Design review of the part built by this model. Coordinates are the model's own, in mm. Coordinates: 2 decimals unless noted, no trailing zeros.
Q1. Take a section at A-A, the plane z = 4. State how many separate pieces and enclosed holes the cut face has, plus the area to 3 significant figures.
Q2. For pin 1 Ø5 at (x, y) = (0, 70.5) entering from -Z, flat-tipped, find the tip position at first contact; note if it passes through.
Q3. For L1, parallel to Y at x = 98, z = 0.9, list the stretches that pass through material, from the lowest coordinate up.
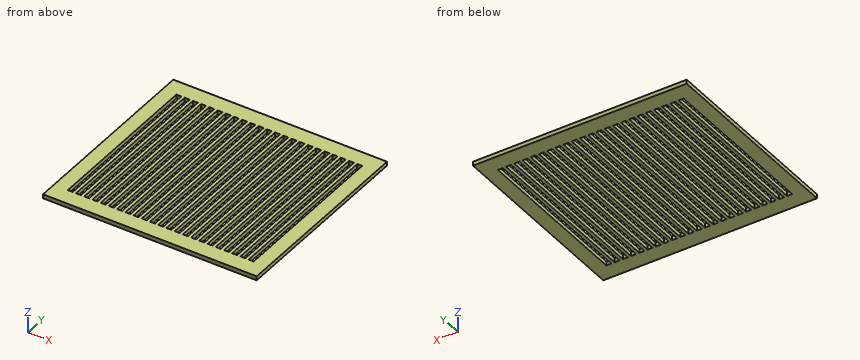
from build123d import *

# Parameters (mm, degrees)
SKETCH_1_W                 = 260
SKETCH_1_H                 = 240
EXTRUDE_1_DEPTH            = 5
SKETCH_2_W                 = 6
SKETCH_2_H                 = 200
CUT_EXTRUDE_1_DEPTH        = 177.988700204
PATTERN_LINEAR_1_COUNT     = 12
PATTERN_LINEAR_1_PITCH     = 10
PATTERN_LINEAR_1_COL_COUNT = 12
PATTERN_LINEAR_1_COL_PITCH = 10


with BuildPart() as part:
    # 草图1 → 凸台-拉伸1 (new body)
    with BuildSketch(Plane.XY):
        Rectangle(SKETCH_1_W, SKETCH_1_H)
    extrude(amount=EXTRUDE_1_DEPTH)

    # 草图2 → 切除-拉伸1 (cut, through all)
    with BuildSketch(Plane.XY.offset(5)):
        Rectangle(SKETCH_2_W, SKETCH_2_H)
    cut_extrude_1 = extrude(amount=-CUT_EXTRUDE_1_DEPTH, mode=Mode.SUBTRACT)

    # 阵列(线性)1: 切除-拉伸1 ×12
    with Locations(*[(i * PATTERN_LINEAR_1_PITCH, 0, 0) for i in range(1, PATTERN_LINEAR_1_COUNT)]):
        add(cut_extrude_1, mode=Mode.SUBTRACT)

    # 阵列(线性)1 col: 切除-拉伸1 ×12
    with Locations(*[(-i * PATTERN_LINEAR_1_COL_PITCH, 0, 0) for i in range(1, PATTERN_LINEAR_1_COL_COUNT)]):
        add(cut_extrude_1, mode=Mode.SUBTRACT)


solid = part.part
Responses:
1. separate pieces: 1
1. enclosed holes: 23
1. area: 34,800 mm2
2. pin 1: passes through
3. L1: y = -120 to -100, 100 to 120
